```python
from build123d import *

# Parameters (mm, degrees)
BOSS_EXTRUDE1_DEPTH                   = 25
BOSS_EXTRUDE1_2_DEPTH                 = 25
SKETCH2_W                             = 5.5
SKETCH2_H                             = 28.1
BOSS_EXTRUDE2_DEPTH                   = 20.3
F_6_0MM_BLIND_DOWEL_HOLE1_D           = 6
F_6_0MM_BLIND_DOWEL_HOLE1_ON_FACE_2_D = 6
F_6_0MM_BLIND_DOWEL_HOLE2_D           = 7
F_6_0MM_BLIND_DOWEL_HOLE2_ON_FACE_2_D = 7


with BuildPart() as part:
    # Sketch1 → Boss-Extrude1 (new, symmetric)
    with BuildSketch(Plane.XY):
        with BuildLine():
            Line((-2.75, 54.931206977), (-2.75, 17.282577933))
            ThreePointArc((-2.75, 17.282577933), (-9.917280768, 14.418652578), (-15.155444566, 8.75))
            Line((-15.155444566, 8.75), (-26.911555625, 15.537393885))
            Line((-26.911555625, 15.537393885), (-11, 28.888774341))
            Line((-11, 28.888774341), (-11, 53.888774341))
            ThreePointArc((-11, 53.888774341), (-6.894729251, 54.566131515), (-2.75, 54.931206977))
        make_face()
    extrude(amount=BOSS_EXTRUDE1_DEPTH, both=True)



with BuildPart() as body_2:
    # Sketch1 → Boss-Extrude1 2 (new, symmetric)
    with BuildSketch(Plane.XY):
        with BuildLine():
            Line((11, 28.888774341), (26.911555625, 15.537393885))
            Line((26.911555625, 15.537393885), (15.155444566, 8.75))
            ThreePointArc((15.155444566, 8.75), (9.917280768, 14.418652578), (2.75, 17.282577933))
            Line((2.75, 17.282577933), (2.75, 54.931206977))
            ThreePointArc((2.75, 54.931206977), (6.894729251, 54.566131515), (11, 53.888774341))
            Line((11, 53.888774341), (11, 28.888774341))
        make_face()
    extrude(amount=BOSS_EXTRUDE1_2_DEPTH, both=True)


with BuildPart() as part_1:
    add(part.part)

    add(body_2.part)  # Boss-Extrude2 merges body 2
    # Sketch2 → Boss-Extrude2 (add, symmetric)
    with BuildSketch(Plane.XY):
        with Locations((0, 36.25)):
            Rectangle(SKETCH2_W, SKETCH2_H)
    extrude(amount=BOSS_EXTRUDE2_DEPTH, both=True)

    # Ø6.0mm Blind Dowel Hole1 (through all)
    with Locations(Plane(origin=(-18.769879496, 22.369071322, 13), x_dir=(0.766044443119, 0.642787609687, 0), z_dir=(-0.642787609687, 0.766044443119, 0))):
        with Locations((0, 0)):
            Hole(F_6_0MM_BLIND_DOWEL_HOLE1_D / 2)

    # Ø6.0mm Blind Dowel Hole1 on face 2 (through all)
    with Locations(Plane(origin=(-18.769879496, 22.369071322, -13), x_dir=(0.766044067841, 0.642788056925, 0), z_dir=(-0.642788056925, 0.766044067841, 0))):
        with Locations((0, 0)):
            Hole(F_6_0MM_BLIND_DOWEL_HOLE1_ON_FACE_2_D / 2)

    # Ø6.0mm Blind Dowel Hole2 (through all)
    with Locations(Plane(origin=(18.769879496, 22.369071322, 13), x_dir=(0.766044443119, -0.642787609687, 0), z_dir=(0.642787609687, 0.766044443119, 0))):
        with Locations((0, 0)):
            Hole(F_6_0MM_BLIND_DOWEL_HOLE2_D / 2)

    # Ø6.0mm Blind Dowel Hole2 on face 2 (through all)
    with Locations(Plane(origin=(18.769879496, 22.369071322, -13), x_dir=(0.766044067841, -0.642788056925, 0), z_dir=(0.642788056925, 0.766044067841, 0))):
        with Locations((0, 0)):
            Hole(F_6_0MM_BLIND_DOWEL_HOLE2_ON_FACE_2_D / 2)


solid = part_1.part
```
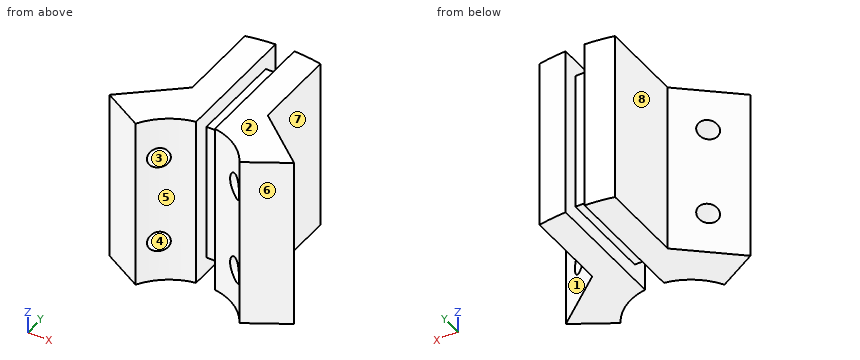
Design review of the part built by this model. Coordinates are the model's own, in mm. Face numbers are marked on the shaded views. A direction names the side the tool comes from. Coordinates: 2 decimals unless noted, no trailing zeros. Loops run counter-clockwise (first coordinate to the right, second up) from the corner with the lowest first, then second, coordinate; pieces in that order, holes last. Notation, with made-up numbers: (30, 4) -> (81, 4) arc R32 cw to (81, 41) -> close; hole circle Ø3 at (2.5, 51.5). An arc over 180 degrees is marked (long way). Answer as a JSON object with one key per item and string values.
Q1. Tool access review of the marked faces 4, 5, 6, 7 and 8: name each direction out of +Z, -Z, +X, -X, +Y, -Y from which nothing blocks a thin tool from reaching the whole face with its end or side.
Answer block:
{"face 4": "none", "face 5": "+Z, -Z, -Y", "face 6": "+Z, -Z, +X, -Y", "face 7": "+Z, -Z, +X, +Y", "face 8": "+Z, -Z, -X, +Y"}
Q2. Take a section at B-B on z = 11. Give the boundary of the cut face in (x, y), plus the area to 3 significant figures.
Answer block:
{"outline": "(-26.91, 15.54) -> (-15.16, 8.75) arc R17.5 cw to (-12.87, 11.86) -> (-20.48, 20.93) -> close; (-17.06, 23.81) -> (-9.44, 14.73) arc R17.5 cw to (-2.75, 17.28) -> (-2.75, 22.2) -> (2.75, 22.2) -> (2.75, 17.28) arc R17.5 cw to (8.9, 15.07) -> (16.57, 24.22) -> (11, 28.89) -> (11, 53.89) arc R55 ccw to (2.75, 54.93) -> (2.75, 50.3) -> (-2.75, 50.3) -> (-2.75, 54.93) arc R55 ccw to (-11, 53.89) -> (-11, 28.89) -> close; (13.3, 11.38) arc R17.5 cw to (15.16, 8.75) -> (26.91, 15.54) -> (20.97, 20.52) -> close", "area": "998 mm^2"}
Q3. Take a section at D-D on x = 22.5. Give the boundary of the cut face in (y, z), plus the area to 3 significant figures.
Answer block:
{"outline": "(12.99, -25) -> (19.24, -25) -> (19.24, 25) -> (12.99, 25) -> close", "area": "312 mm^2"}
Q4. Take a section at C-C on z = -18. Give the boundary of the cut face in (x, y).
Answer block:
{"outline": "(-26.91, 15.54) -> (-15.16, 8.75) arc R17.5 cw to (-2.75, 17.28) -> (-2.75, 22.2) -> (2.75, 22.2) -> (2.75, 17.28) arc R17.5 cw to (15.16, 8.75) -> (26.91, 15.54) -> (11, 28.89) -> (11, 53.89) arc R55 ccw to (2.75, 54.93) -> (2.75, 50.3) -> (-2.75, 50.3) -> (-2.75, 54.93) arc R55 ccw to (-11, 53.89) -> (-11, 28.89) -> close"}
Q5. The part is to be moulded in two halves that separate along Z. For the marked faces 1, 2 and 3, say which applies: +Z half, -Z half, draft (parallel to the pull), parting line (faces both ways), or undercut.
Answer block:
{"face 1": "draft", "face 2": "+Z half", "face 3": "undercut"}
Q6. Take a section at A-A on y = 31. Give the boundary of the cut face in (x, z).
Answer block:
{"outline": "(-11, -25) -> (-2.75, -25) -> (-2.75, -20.3) -> (2.75, -20.3) -> (2.75, -25) -> (11, -25) -> (11, 25) -> (2.75, 25) -> (2.75, 20.3) -> (-2.75, 20.3) -> (-2.75, 25) -> (-11, 25) -> close"}
Q7. Clearance check with flat-ended pins moving along their axes: pin 1 Ø1.5 at (y, z) = (49, 13.5) entering from -X; pin 2 Ø11.5 at (y, z) = (40.5, 9) entering from +X; pin 3 Ø1.5 at (x, z) = (9, 16.5) entering from +Y. State where each tip first meets the part, or that it passes through.
Answer block:
{"pin 1": "stops at x = -11", "pin 2": "stops at x = 11", "pin 3": "stops at y = 54.38"}
Q8. To check wall thickness, follow L1, parallel to Z at x = 18, y = 21.5; L2, parallel to X at y = 19.5, z = 11; L3, parallel to X at y = 52, z = 10.5. State the ranges of each line that lie inside material, in increasing order.
Answer block:
{"L1": "z = -25 to -16.5, -9.5 to 9.5, 16.5 to 25", "L2": "x = -22.19 to -19.28, -13.44 to -2.75, 2.75 to 12.61, 20.11 to 22.19", "L3": "x = -11 to -2.75, 2.75 to 11"}
